Source: three-view drawing plus pictorial views. Frame: mm from the lowest corner of the part. A direction names the side the tool comes from. Give positions to 0.01 mm unless a question says otherwise; leave off trailing zeros. Write each loop counter-clockwise with the first axis right and the second up, starting at its lowest first coordinate (ties: lowest second). Pieces come first, ordered by that corner, then holes. Notation, with made-up numbers: (13, 47) -> (44, 47) arc R18 cw to (44, 71) -> close; hole circle Ø3 at (-33.5, -20). An arc over 180 degrees is marked (long way). Answer in a Markdown table with one row per item. Add a question column.
Item 1: First-contact query: P1, Ø3, axis at x = 5, y = 1.5, coming from the -Z side; P2, Ø6, axis at x = 5.5, z = 3, coming from the +Y side; P3, Ø2, axis at x = 3.5, z = 8.5, coming from the -Y side (1 decimal). Flat tips, straight axial feed; report the tip coordinate or a pass-through.
Item 2: Draft query along Y for the marked faces 1, 2, 3 and 4. Return one class per face: +Y half, -Y half, draft (parallel to the pull), parting line (faces both ways), or undercut.
Item 3: Access query for the marked faces 5 and 6. Directions: +Z, -Z, +X, -X, +Y, -Y. A direction counts if a zero-diameter tool reaches every point of the face in a straight line with its end or side. Return the directions, or none.
Item 4: Material intervals for probe 1 along Z at (x, y) = (0.5, 5); probe 2 along X at (y, z) = (1.5, 9.75) (1 decimal); probe 3 along X at (y, z) = (7.25, 6.25) (1 decimal), sorted ascending. Write a range as from..to.
Item 5: Section query A-A on z = 8.25. Output: boundary loops of the cut face in (x, y).
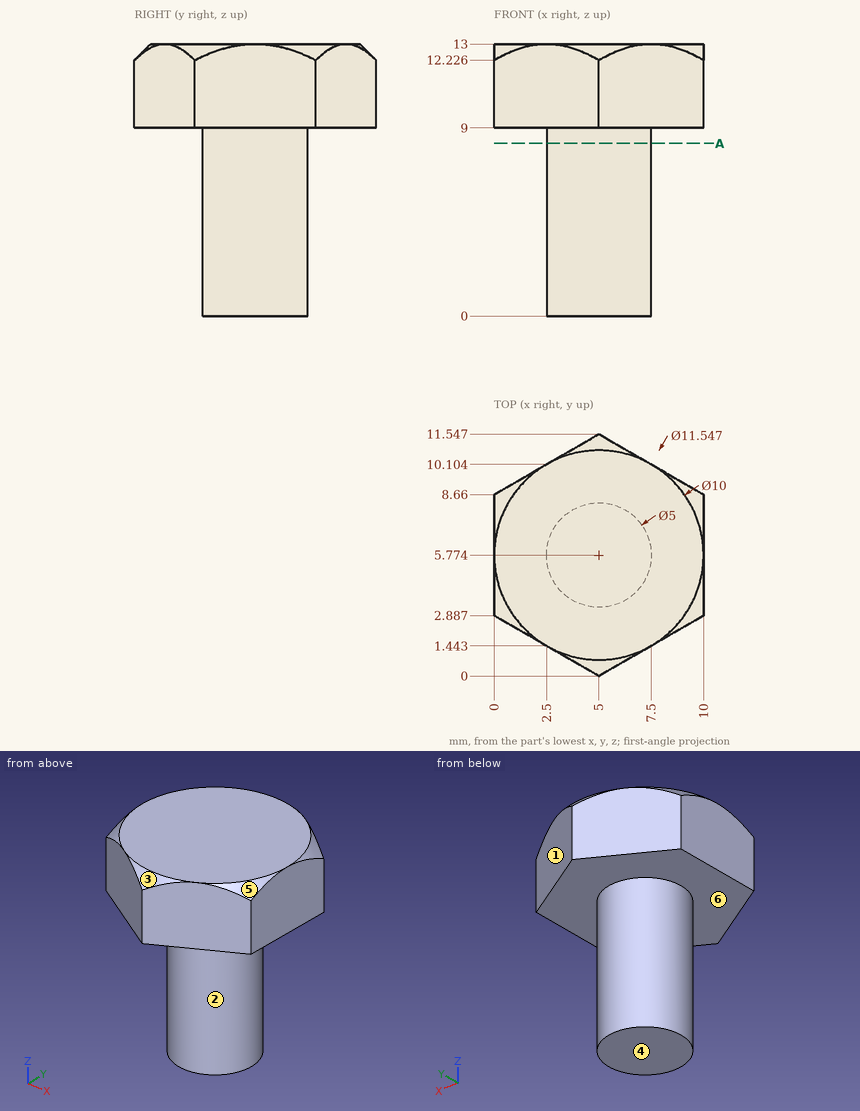
Findings below:
| question | item | result |
|---|---|---|
| 1 | P1 | stops at z = 9 |
| 1 | P2 | stops at y = 8.27 |
| 1 | P3 | stops at y = 0.4 |
| 2 | face 1 | +Y half |
| 2 | face 2 | parting line |
| 2 | face 3 | -Y half |
| 2 | face 4 | draft |
| 3 | face 5 | +Z, +X, -Y |
| 3 | face 6 | -Z |
| 4 | probe 1 | z = 9..13 |
| 4 | probe 2 | x = 2.4..7.6 |
| 4 | probe 3 | x = 3..7 |
| 5 | outline | circle Ø5 at (5, 5.77) |
